The listing builds one solid part. Answer for the finished solid, in the listing's coordinates (mm). Face numbers are marked on the shaded views. Give positions to 0.01 mm unless a question says otherwise; leave off trailing zeros. Order: outer loops, then holes, each group sorted by start corner. A loop starts at its lowest first (then second) coordinate and runs counter-clockwise, first axis right, second up. Notation, with made-up numbers: (17.5, 69.5) - (43.5, 69.5) arc R11 cw to (43.5, 79.5) - close; hole circle Ø10 at (34, 25.25). An arc over 180 degrees is marked (long way). Answer in a Markdown table with one row per item.
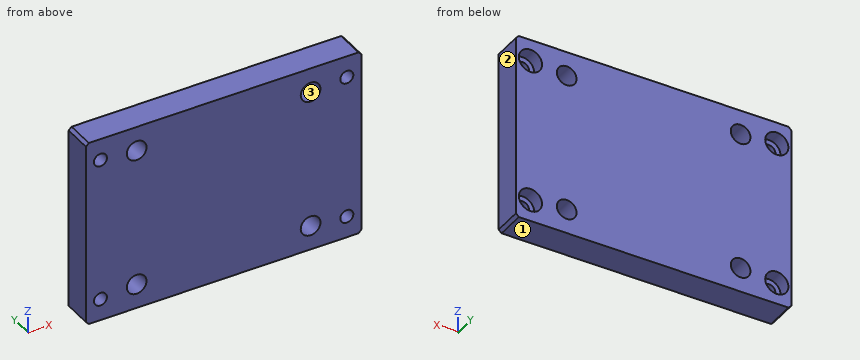
from build123d import *

# Parameters (mm, degrees)
SKETCH_1_W                   = 95
SKETCH_1_H                   = 65
EXTRUDE_1_DEPTH              = 5
CHAMFER_1_SIZE               = 1
HOLE_WIZARD_M4_1_D           = 4.5
HOLE_WIZARD_M4_1_CBORE_D     = 8
HOLE_WIZARD_M4_1_CBORE_DEPTH = 4.6
HOLE_WIZARD_M8_1_D           = 6.8


with BuildPart() as part:
    # 草图1 → 凸台-拉伸1 (new, symmetric)
    with BuildSketch(Plane(origin=(0, 0, 0), x_dir=(1, 0, 0), z_dir=(0, 1, 0))):
        Rectangle(SKETCH_1_W, SKETCH_1_H)
    extrude(amount=EXTRUDE_1_DEPTH, both=True)

    # 倒角1
    chamfer_1_edges = [part.edges().sort_by_distance(p)[0] for p in [
        (47.5, 0, 32.5),
        (-47.5, 0, 32.5),
        (-47.5, 0, -32.5),
        (47.5, 0, -32.5),
    ]]
    chamfer(chamfer_1_edges, length=CHAMFER_1_SIZE)

    # M4 六角圆柱头螺钉的柱形沉头孔1 (through all)
    with Locations(Plane(origin=(0, 5, 0), x_dir=(1, 0, 0), z_dir=(0, 1, 0))):
        with Locations((-42.5, 25), (-42.5, -25), (42.5, -25), (42.5, 25)):
            CounterBoreHole(HOLE_WIZARD_M4_1_D / 2, HOLE_WIZARD_M4_1_CBORE_D / 2, HOLE_WIZARD_M4_1_CBORE_DEPTH)

    # M8 螺纹孔1 (through all)
    with Locations(Plane(origin=(0, 5, 0), x_dir=(1, 0, 0), z_dir=(0, 1, 0))):
        with Locations((30, 24), (30, -24), (-30, -24), (-30, 24)):
            Hole(HOLE_WIZARD_M8_1_D / 2)


solid = part.part
Item 1: Determine the mould class of the marked faces 1, 2 and 3 for opening direction X: pulls with the +X half, pulls with the -X half, needs draft (parallel to the pull), parting line crosses it, or undercut.
Answer block:
| item | result |
|---|---|
| face 1 | needs draft |
| face 2 | pulls with the +X half |
| face 3 | undercut |
Item 2: Find section A-A on x = 42.5. Write down the section's boundary in (y, z), then the cut area to 3 significant figures.
Answer block:
| item | result |
|---|---|
| outline | (-5, -32.5) - (5, -32.5) - (5, -29) - (0.4, -29) - (0.4, -27.25) - (-5, -27.25) - close; (-5, -22.75) - (0.4, -22.75) - (0.4, -21) - (5, -21) - (5, 21) - (0.4, 21) - (0.4, 22.75) - (-5, 22.75) - close; (-5, 27.25) - (0.4, 27.25) - (0.4, 29) - (5, 29) - (5, 32.5) - (-5, 32.5) - close |
| area | 528 mm² |
Item 3: Find section D-D on x = -30. Write down the section's boundary in (y, z), then the cut area to 3 significant figures.
Answer block:
| item | result |
|---|---|
| outline | (-5, -32.5) - (5, -32.5) - (5, -27.4) - (-5, -27.4) - close; (-5, -20.6) - (5, -20.6) - (5, 20.6) - (-5, 20.6) - close; (-5, 27.4) - (5, 27.4) - (5, 32.5) - (-5, 32.5) - close |
| area | 514 mm² |
Item 4: Each of these flat-tipped pins is pushed along its axis until it touches: P1, Ø8, axis at x = 30, z = -24, coming from the +Y side; P2, Ø3.5, axis at x = 42.5, z = 25, coming from the -Y side; P3, Ø7, axis at x = 42.5, z = 25, coming from the +Y side. Where does it stop, or does it pass through?
Answer block:
| item | result |
|---|---|
| P1 | y = 5 |
| P2 | through |
| P3 | y = 0.4 |
Item 5: Consider line 1 (Z direction, x = -42.5, y = 2.6); line 2 (Z direction, x = 30, y = 0.75); line 3 (X direction, y = 2.25, z = 22.5). Determine where each line is inside the solid, lowest interval first.
Answer block:
| item | result |
|---|---|
| line 1 | -32.5 to -29, -21 to 21, 29 to 32.5 |
| line 2 | -32.5 to -27.4, -20.6 to 20.6, 27.4 to 32.5 |
| line 3 | -47.5 to -45.62, -39.38 to -33.05, -26.95 to 26.95, 33.05 to 39.38, 45.62 to 47.5 |
Item 6: Find section C-C on z = -25. Write down the section's boundary in (x, y), then the cut area to 3 significant figures.
Answer block:
| item | result |
|---|---|
| outline | (-47.5, -5) - (-44.75, -5) - (-44.75, 0.4) - (-46.5, 0.4) - (-46.5, 5) - (-47.5, 5) - close; (-40.25, -5) - (-33.25, -5) - (-33.25, 5) - (-38.5, 5) - (-38.5, 0.4) - (-40.25, 0.4) - close; (-26.75, -5) - (26.75, -5) - (26.75, 5) - (-26.75, 5) - close; (33.25, -5) - (40.25, -5) - (40.25, 0.4) - (38.5, 0.4) - (38.5, 5) - (33.25, 5) - close; (44.75, -5) - (47.5, -5) - (47.5, 5) - (46.5, 5) - (46.5, 0.4) - (44.75, 0.4) - close |
| area | 698 mm² |
Item 7: Find section B-B on y = -3. Count the separate pieces of the cut face and the enclosed holes in it, then the cut area to 3 significant figures.
Answer block:
| item | result |
|---|---|
| separate pieces | 1 |
| enclosed holes | 8 |
| area | 5,960 mm² |
